Can you work these out from the drawing? Everything is in mm from the part's minimum corner. Round coordinates to 2 decimals unless told otherwise and drop trailing zeros. Loops run counter-clockwise (first coordinate to the right, second up) from the corner with the lowest first, then second, coordinate; pieces in that order, holes last. Notation, with made-up numbers: (-6.75, 48.5) - (19.25, 48.5) arc R24 cw to (19.25, 77.5) - close; hole circle Ø4 at (-24, 24). An arc over 180 degrees is marked (long way). Answer as a JSON object with one key per item and string values. Group by question number.
1) If I drill on line 1 along Y through (x, z) = (29.5, 2); line 2 along X through (y, z) = (3, 6.25); line 3 along Y through (x, z) = (37.5, 10.75), over which ranges is the centre line in solid material (lowest first)? Write a range as [from, to].
2) I want a section at B-B, the plane z = 13.75. Please give me the cut outline in (x, y), then the cut area to 3 significant figures.
3) I want a section at A-A, the plane y = 32. Please give me the cut outline in (x, z).
4) Will this pin go through, and if not, where does the flat tip stop? P1, Ø8, axis at y = 26.5, z = 11.5, coming from the -X side.
5) I want a section at C-C, the plane x = 7. Please give me the cut outline in (y, z), then the cut area to 3 significant figures.
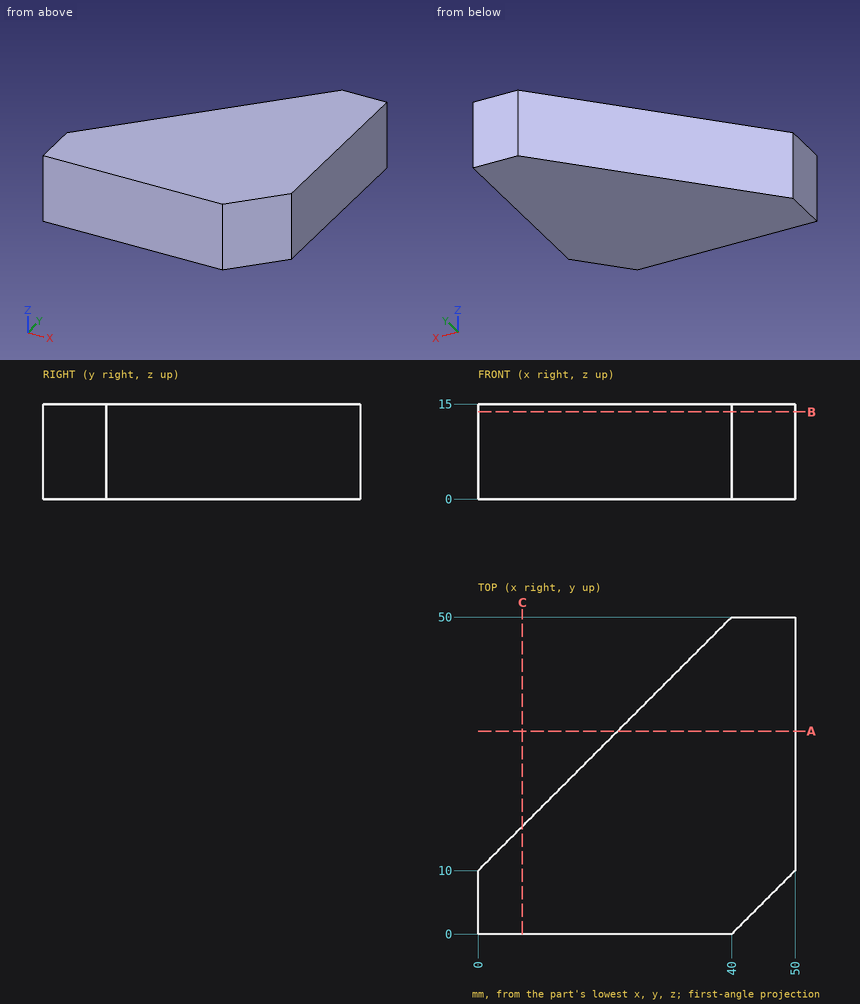
Outcome:
{
 "1": {"line 1": "[0, 39.5]", "line 2": "[0, 43]", "line 3": "[0, 47.5]"},
 "2": {"outline": "(0, 0) - (40, 0) - (50, 10) - (50, 50) - (40, 50) - (0, 10) - close", "area": "1,650 mm^2"},
 "3": {"outline": "(22, 0) - (50, 0) - (50, 15) - (22, 15) - close"},
 "4": {"P1": "x = 12.5"},
 "5": {"outline": "(0, 0) - (17, 0) - (17, 15) - (0, 15) - close", "area": "255 mm^2"}
}
